Here's the drawing with two shaded views (mm, measured from the low corner). I have some questions. Round coordinates to 2 decimals unless told otherwise and drop trailing zeros. Write each loop counter-clockwise with the first axis right and the second up, starting at its lowest first coordinate (ties: lowest second). Pieces come first, ordered by that corner, then holes. Notation, with made-up numbers: M 76.5,82.25 L 121.5,82.25 A22 ccw 121.5,93.25 Z; hole C 58,34 d4. An arc over 180 degrees is marked long. Write item = value, one per line. Start each with the question number.
(1) I want a section at A-A (z = 20.5). List the corners of the cut face in (x, y) for me, and give its area (3 significant figures).
(2) I want a section at B-B (y = 21.5). List the corners of the cut face in (x, z) for me.
(3) Will these pins go through, and if not, where does the flat tip stop? pin 1 Ø2 at (x, z) = (26, 37.5) entering from +Y; pin 2 Ø1.5 at (y, z) = (10, 79.5) entering from -X.
(4) I need wall thicknesses on line 1 along X through (y, z) = (6.25, 87); line 2 along Y through (x, z) = (19.75, 59). Which ranges of each line are inside material? Lowest first, please.
(5) If we mould it in two halves opening along Y, with no side actions, what happens to the marked faces 1, 2 and 3? For each: released by +Y, released by -Y, zero draft, split by the parting line, or undercut.
(6) I want a section at C-C (x = 25.5). List the corners of the cut face in (y, z) for me, and give its area (3 significant figures).
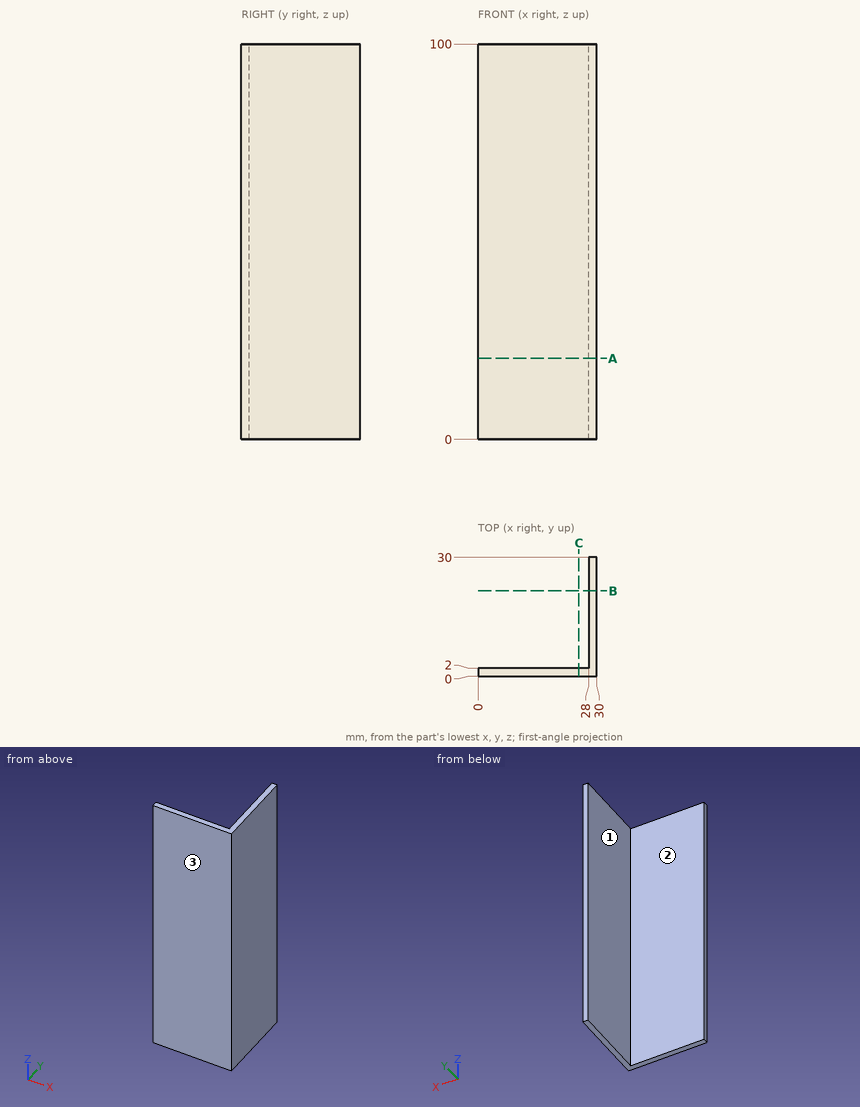
Returned:
q1.outline = M 0,0 L 30,0 L 30,30 L 28,30 L 28,2 L 0,2 Z
q1.area = 116 mm²
q2.outline = M 28,0 L 30,0 L 30,100 L 28,100 Z
q3.pin_1 = 2
q3.pin_2 = 28
q4.line_1 = 28 to 30
q4.line_2 = 0 to 2
q5.face_1 = zero draft
q5.face_2 = released by +Y
q5.face_3 = released by -Y
q6.outline = M 0,0 L 2,0 L 2,100 L 0,100 Z
q6.area = 200 mm²
